```python
from build123d import *

# Parameters (mm, degrees)
BASE_BRACKET_80MM_DEPTH   = 40
UPPER_LUG_PLATE_DEPTH     = 10
SKETCH2_3_R               = 20
SKETCH2_3_R_2             = 10
UPPER_LUG_HUB_DEPTH       = 25
FRONT_LUG_PROFILE_R       = 25
FRONT_LUG_PROFILE_R_2     = 15
FRONT_LUG_BOSS_DEPTH      = 10
FRONT_LUG_BORE_REACH      = 150.661
SKETCH4_2_R               = 15
CONNECTING_WEB_DEPTH      = 5
WEB_PAD_A_PROFILE_W       = 10
WEB_PAD_A_PROFILE_H       = 10
WEB_PAD_A_DEPTH           = 5
WEB_PAD_B_PROFILE_W       = 10
WEB_PAD_B_PROFILE_H       = 50
WEB_PAD_B_DEPTH           = 5
WEB_RELIEF_CUT_REACH      = 152.083
WEB_RELIEF_PROFILE_W      = 35
WEB_RELIEF_PROFILE_H      = 5
WEB_RELIEF_FILLET_R10_R   = 10
GUSSET_RIB_DEPTH          = 5
RIB_TRIM_CUT_REACH        = 113.467
RIB_PAD_A_DEPTH           = 5
RIB_PAD_B_DEPTH           = 5
LUG_CLEARANCE_CUT_REACH   = 154.971
RIB_NOTCH_CUT_DEPTH       = 10
UPPER_HUB_BORE_20_REACH   = 109.703
UPPER_HUB_BORE_PROFILE_R  = 10
BASE_ARC_CUTOUT_REACH     = 142
BASE_ARC_CUTOUT_PROFILE_R = 20


with BuildPart() as part:
    # Base Bracket Profile → Base Bracket 80mm (new, symmetric)
    with BuildSketch(Plane(origin=(0, 0, 0), x_dir=(0, 0, -1), z_dir=(1, 0, 0))):
        Polygon((0, 0), (60, 0), (60, 10), (10, 10), (10, 70), (50, 70), (50, 80), (0, 80), align=None)
    extrude(amount=BASE_BRACKET_80MM_DEPTH, both=True)

    # Upper Lug Profile → Upper Lug Plate (add)
    with BuildSketch(Plane(origin=(0, 0, -50), x_dir=(-1, 0, 0), z_dir=(0, 0, -1))):
        with BuildLine():
            Line((-40, 80), (0, 80))
            Line((0, 80), (0, 90))
            ThreePointArc((0, 90), (-17.281273745, 99.932349938), (-17.398181668, 119.864242224))
            Line((-17.398181668, 119.864242224), (-40, 80))
        make_face()
        with BuildLine():
            Line((0, 90), (0, 80))
            Line((0, 80), (40, 80))
            Line((40, 80), (17.398181668, 119.864242224))
            ThreePointArc((17.398181668, 119.864242224), (19.338609482, 115.100802223), (20, 110))
            ThreePointArc((20, 110), (14.142135624, 95.857864376), (0, 90))
        make_face()
    extrude(amount=-UPPER_LUG_PLATE_DEPTH)

    # Sketch2_3 → Upper Lug Hub (add)
    with BuildSketch(Plane(origin=(0, 0, -50), x_dir=(-1, 0, 0), z_dir=(0, 0, -1))):
        with Locations((0, 110)):
            Circle(SKETCH2_3_R)
        with Locations((0, 110)):
            Circle(SKETCH2_3_R_2, mode=Mode.SUBTRACT)
    extrude(amount=-UPPER_LUG_HUB_DEPTH)

    # Front Lug Profile → Front Lug Boss (add)
    with BuildSketch(Plane.XY):
        with Locations((0, 40)):
            Circle(FRONT_LUG_PROFILE_R)
        with Locations((0, 40)):
            Circle(FRONT_LUG_PROFILE_R_2, mode=Mode.SUBTRACT)
    extrude(amount=FRONT_LUG_BOSS_DEPTH)

    # Sketch4_2 → Front Lug Bore (cut, up to next)
    with BuildSketch(Plane.XY, mode=Mode.PRIVATE) as front_lug_bore_sk1:
        with Locations((0, 40)):
            Circle(SKETCH4_2_R)
    front_lug_bore_tool1 = extrude(front_lug_bore_sk1.sketch, amount=-FRONT_LUG_BORE_REACH, mode=Mode.PRIVATE) & part.part
    add(front_lug_bore_tool1.solids().sort_by_distance((0, 40, 0))[0], mode=Mode.SUBTRACT)



with BuildPart() as body_2:
    # Connecting Web Profile → Connecting Web (new, symmetric)
    with BuildSketch(Plane(origin=(0, 0, 0), x_dir=(0, 0, -1), z_dir=(1, 0, 0))):
        Polygon((-10, 66.461599877), (-10, 90), (40, 90), (40, 80), (0, 80), (0, 66.461599877), align=None)
    extrude(amount=CONNECTING_WEB_DEPTH, both=True)


with BuildPart() as body_3:
    # Web Pad A Profile → Web Pad A (new, symmetric)
    with BuildSketch(Plane.XZ.offset(-66.461599877)):
        with Locations((0, 5)):
            Rectangle(WEB_PAD_A_PROFILE_W, WEB_PAD_A_PROFILE_H)
    extrude(amount=WEB_PAD_A_DEPTH, both=True)


with BuildPart() as part_1:
    add(part.part)

    add(body_2.part)  # Web Pad B merges body 2
    # Web Pad B Profile → Web Pad B (add, symmetric)
    with BuildSketch(Plane(origin=(0, 90, 0), x_dir=(1, 0, 0), z_dir=(0, 1, 0))):
        with Locations((0, 15)):
            Rectangle(WEB_PAD_B_PROFILE_W, WEB_PAD_B_PROFILE_H)
    extrude(amount=WEB_PAD_B_DEPTH, both=True)

    # Combine Web Pads: union body 3
    add(body_3.part)

    # Web Relief Profile → Web Relief Cut (cut, up to next)
    with BuildSketch(Plane(origin=(5, 0, 0), x_dir=(0, 0, -1), z_dir=(1, 0, 0)), mode=Mode.PRIVATE) as web_relief_cut_sk1:
        with Locations((7.5, 92.5)):
            Rectangle(WEB_RELIEF_PROFILE_W, WEB_RELIEF_PROFILE_H)
    web_relief_cut_tool1 = extrude(web_relief_cut_sk1.sketch, amount=-WEB_RELIEF_CUT_REACH, mode=Mode.PRIVATE) & part_1.part
    add(web_relief_cut_tool1.solids().sort_by_distance((5, 92.5, -7.5))[0], mode=Mode.SUBTRACT)

    # Web Relief Fillet R10
    web_relief_fillet_r10_edges = [part_1.edges().sort_by_distance(p)[0] for p in [
        (0, 90, 10),
    ]]
    fillet(web_relief_fillet_r10_edges, radius=WEB_RELIEF_FILLET_R10_R)

    # Gusset Rib Path → Gusset Rib (add, symmetric)
    with BuildSketch(Plane(origin=(0, 40, 0), x_dir=(-1, 0, 0), z_dir=(0, -1, 0))):
        Polygon((-25, -10), (-40, 0), (-34.452998038, 8.320502943), (-19.452998038, -1.679497057), align=None)
    gusset_rib = extrude(amount=GUSSET_RIB_DEPTH, both=True)

    # Rib Trim Profile → Rib Trim Cut (cut, up to next)
    with BuildSketch(Plane(origin=(0, 45, 0), x_dir=(1, 0, 0), z_dir=(0, 1, 0)), mode=Mode.PRIVATE) as rib_trim_cut_sk1:
        Polygon((24.494897428, -10), (40, 0), (25, -10), align=None)
    rib_trim_cut_tool1 = extrude(rib_trim_cut_sk1.sketch, amount=-RIB_TRIM_CUT_REACH, mode=Mode.PRIVATE) & part_1.part
    rib_trim_cut = rib_trim_cut_tool1.solids().sort_by_distance((29.831632, 45, 6.666667))[0]
    add(rib_trim_cut, mode=Mode.SUBTRACT)

    # Rib Pad A Profile → Rib Pad A (add, symmetric)
    with BuildSketch(Plane(origin=(12.692307692, 0, -8.461538462), x_dir=(0.5547001962252294, 0, 0.8320502943378436), z_dir=(-0.8320502943378436, 0, 0.5547001962252294))):
        with BuildLine():
            Line((21.277421237, 35), (21.91421024, 35))
            Line((21.91421024, 35), (21.91421024, 37.248507099))
            add(Edge.make_bspline(
                [(21.277421237, 35), (21.688173728, 36.116205467), (21.91421024, 37.248507099)],
                knots=[2.940234733, 2.940234733, 2.940234733, 3.031309523, 3.031309523, 3.031309523], degree=2, weights=[1, 0.998963352, 1]))
        make_face()
    rib_pad_a = extrude(amount=RIB_PAD_A_DEPTH, both=True)

    # Rib Pad B Profile → Rib Pad B (add, symmetric)
    with BuildSketch(Plane(origin=(12.692307692, 0, -8.461538462), x_dir=(0.5547001962252294, 0, 0.8320502943378436), z_dir=(-0.8320502943378436, 0, 0.5547001962252294))):
        with BuildLine():
            Line((21.91421024, 42.751492901), (21.91421024, 45))
            Line((21.91421024, 45), (21.277421237, 45))
            add(Edge.make_bspline(
                [(21.91421024, 42.751492901), (21.688173728, 43.883794533), (21.277421237, 45)],
                knots=[3.251875784, 3.251875784, 3.251875784, 3.342950574, 3.342950574, 3.342950574], degree=2, weights=[1, 0.998963352, 1]))
        make_face()
    rib_pad_b = extrude(amount=RIB_PAD_B_DEPTH, both=True)

    # Lug Clearance Cut: up to this plane
    lug_clearance_cut_end = Plane(origin=(20.687872941, 35, 12.5456876), z_dir=(-0.5547001962252294, 0, -0.8320502943378436))
    # Lug Clearance Profile → Lug Clearance Cut (cut, up to the surface)
    with BuildSketch(Plane.XY.offset(10), mode=Mode.PRIVATE) as lug_clearance_cut_sk1:
        with BuildLine():
            Line((24.494897428, 37.216718732), (24.494897428, 35))
            ThreePointArc((24.494897428, 35), (-17.67766953, 22.32233047), (-5, 64.494897428))
            Line((-5, 64.494897428), (-5, 80))
            Line((-5, 80), (5, 80))
            Line((5, 80), (5, 64.494897428))
            ThreePointArc((5, 64.494897428), (17.67766953, 57.67766953), (24.494897428, 45))
            Line((24.494897428, 45), (24.494897428, 37.216718732))
        make_face()
    lug_clearance_cut_tool1 = split(extrude(lug_clearance_cut_sk1.sketch, amount=LUG_CLEARANCE_CUT_REACH, mode=Mode.PRIVATE), bisect_by=lug_clearance_cut_end, keep=Keep.BOTH, mode=Mode.PRIVATE)
    lug_clearance_cut = lug_clearance_cut_tool1.solids().sort_by_distance((-0.039461, 42.32819, 10))[0]
    add(lug_clearance_cut, mode=Mode.SUBTRACT)

    # Rib Notch Profile → Rib Notch Cut (cut)
    with BuildSketch(Plane.XZ.offset(-35)):
        Polygon((24.848124412, 9.772186619), (24.494897428, 10), (24.494897428, 10.007671275), align=None)
    rib_notch_cut = extrude(amount=-RIB_NOTCH_CUT_DEPTH, mode=Mode.SUBTRACT)

    # Rib Features Mirror: Gusset Rib, Rib Trim Cut, Rib Pad A, Rib Pad B, Lug Clearance Cut, Rib Notch Cut across plane
    add(gusset_rib.mirror(Plane(origin=(0, 0, 0), x_dir=(0, 0, 1), z_dir=(1, 0, 0))))
    add(rib_trim_cut.mirror(Plane(origin=(0, 0, 0), x_dir=(0, 0, 1), z_dir=(1, 0, 0))), mode=Mode.SUBTRACT)
    add(rib_pad_a.mirror(Plane(origin=(0, 0, 0), x_dir=(0, 0, 1), z_dir=(1, 0, 0))))
    add(rib_pad_b.mirror(Plane(origin=(0, 0, 0), x_dir=(0, 0, 1), z_dir=(1, 0, 0))))
    add(lug_clearance_cut.mirror(Plane(origin=(0, 0, 0), x_dir=(0, 0, 1), z_dir=(1, 0, 0))), mode=Mode.SUBTRACT)
    add(rib_notch_cut.mirror(Plane(origin=(0, 0, 0), x_dir=(0, 0, 1), z_dir=(1, 0, 0))), mode=Mode.SUBTRACT)

    # Upper Hub Bore Profile → Upper Hub Bore _20 (cut, up to next)
    with BuildSketch(Plane(origin=(0, 80, 0), x_dir=(1, 0, 0), z_dir=(0, 1, 0)), mode=Mode.PRIVATE) as upper_hub_bore_20_sk1:
        with Locations(Location((-20, 25, 0), (0, 0, 270))):
            Circle(UPPER_HUB_BORE_PROFILE_R)
    upper_hub_bore_20_tool1 = extrude(upper_hub_bore_20_sk1.sketch, amount=-UPPER_HUB_BORE_20_REACH, mode=Mode.PRIVATE) & part_1.part
    # Upper Hub Bore Profile → Upper Hub Bore _20 (cut, up to next)
    with BuildSketch(Plane(origin=(0, 80, 0), x_dir=(1, 0, 0), z_dir=(0, 1, 0)), mode=Mode.PRIVATE) as upper_hub_bore_20_sk2:
        with Locations(Location((20, 25, 0), (0, 0, 270))):
            Circle(UPPER_HUB_BORE_PROFILE_R)
    upper_hub_bore_20_tool2 = extrude(upper_hub_bore_20_sk2.sketch, amount=-UPPER_HUB_BORE_20_REACH, mode=Mode.PRIVATE) & part_1.part
    add(upper_hub_bore_20_tool1.solids().sort_by_distance((-20, 80, -25))[0], mode=Mode.SUBTRACT)
    add(upper_hub_bore_20_tool2.solids().sort_by_distance((20, 80, -25))[0], mode=Mode.SUBTRACT)

    # Base Arc Cutout Profile → Base Arc Cutout (cut, up to next)
    with BuildSketch(Plane(origin=(0, 10, 0), x_dir=(1, 0, 0), z_dir=(0, 1, 0)), mode=Mode.PRIVATE) as base_arc_cutout_sk1:
        with Locations((0, 60)):
            Circle(BASE_ARC_CUTOUT_PROFILE_R)
    base_arc_cutout_tool1 = extrude(base_arc_cutout_sk1.sketch, amount=-BASE_ARC_CUTOUT_REACH, mode=Mode.PRIVATE) & part_1.part
    add(base_arc_cutout_tool1.solids().sort_by_distance((0, 10, -60))[0], mode=Mode.SUBTRACT)


solid = part_1.part
```
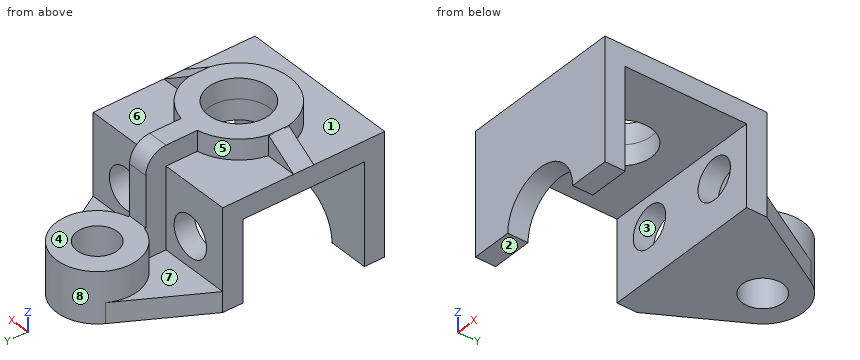
Part model, mm, in its own coordinate system. Face numbers are marked on the shaded views. A direction names the side the tool comes from. Round coordinates to 2 decimals unless told otherwise and drop trailing zeros. Loops run counter-clockwise (first coordinate to the right, second up) from the corner with the lowest first, then second, coordinate; pieces in that order, holes last. Notation, with made-up numbers: (30.25, 16) -> (60.25, 16) arc R26 ccw to (60.25, 47) -> close; hole circle Ø6 at (0.5, -22.75). An arc over 180 degrees is marked (long way). Use a Markdown table: item, result.
1) Cut at D-D, the plane x = -22. List the corners of the cut face in (y, z).
The answers:
| item | result |
|---|---|
| outline | (0, -60) -> (10, -60) -> (10, -10) -> (70, -10) -> (70, -15.2) -> (80, -15.2) -> (80, 0) -> (51.87, 0) -> (51.87, 10) -> (28.13, 10) -> (28.13, 0) -> (0, 0) -> close; (70, -50) -> (111.75, -50) -> (111.75, -40) -> (80, -40) -> (80, -34.8) -> (70, -34.8) -> close |
2) Probe line 1 (Y direction, x = 0, z = -37.75); line 2 (Y direction, x = 17, z = -12); line 3 (X direction, y = 73.5, z = -25). List the from-to ranges inside material, lowest first. Write a range as [from, to].
The answers:
| item | result |
|---|---|
| line 1 | y = [0, 10], [70, 100], [120, 130] |
| line 2 | y = [0, 10], [70, 80] |
| line 3 | x = [-40, -30], [-10, 10], [30, 40] |
3) Cut at C-C, the plane z = -53.5. List the corners of the cut face in (x, y), and give its area (3 significant figures).
The answers:
| item | result |
|---|---|
| outline | (-40, 0) -> (-18.91, 0) -> (-18.91, 10) -> (-40, 10) -> close; (18.91, 0) -> (40, 0) -> (40, 10) -> (18.91, 10) -> close |
| area | 422 mm2 |
4) Pull direction Z, two halves, no side cores. Call the marked faces 1, 2 and 3: pulls with the +Z half, pulls with the -Z half, needs draft (parallel to the pull), parting line crosses it, or undercut.
The answers:
| item | result |
|---|---|
| face 1 | pulls with the +Z half |
| face 2 | pulls with the -Z half |
| face 3 | undercut |
5) Tool access for the marked faces 4, 5, 6, 7 and 8: list every direction of +Z, -Z, +X, -X, +Y, -Y with a clear straight run to the whole face (end or side of a thin tool).
The answers:
| item | result |
|---|---|
| face 4 | +Z, +X, -X, +Y |
| face 5 | +Z, -X, +Y |
| face 6 | +Z, +X, +Y |
| face 7 | +Z, -X |
| face 8 | +Z |
6) Drop flat-ended pins along their axis: pin 1 Ø3 at (x, y) = (-15.5, 17.5) entering from +Z; pin 2 Ø5 at (x, z) = (34, 7) entering from -Y; pin 3 Ø17.5 at (x, y) = (20.5, 110) entering from +Z; pin 4 Ø12 at (x, y) = (16, 25.5) entering from -Z. Give the stop position or say it passes through.
The answers:
| item | result |
|---|---|
| pin 1 | stops at z = 0 |
| pin 2 | passes through |
| pin 3 | stops at z = -25 |
| pin 4 | stops at z = -10 |
7) Cut at A-A, the plane y = 40. List the corners of the cut face in (x, z).
The answers:
| item | result |
|---|---|
| outline | (-40, -10) -> (-15, -10) -> (-15, 10) -> (-24.49, 10) -> (-40, 0) -> close; (15, -10) -> (40, -10) -> (40, 0) -> (24.49, 10) -> (15, 10) -> close |
8) Cut at B-B, the plane x = 0. List the corners of the cut face in (y, z).
The answers:
| item | result |
|---|---|
| outline | (0, -40) -> (10, -40) -> (10, -10) -> (25, -10) -> (25, 10) -> (15, 10) -> (15, 0) -> (0, 0) -> close; (55, -10) -> (70, -10) -> (70, -50) -> (100, -50) -> (100, -25) -> (90, -25) -> (90, 0) arc R10 ccw to (80, 10) -> (55, 10) -> close; (120, -50) -> (130, -50) -> (130, -25) -> (120, -25) -> close |
